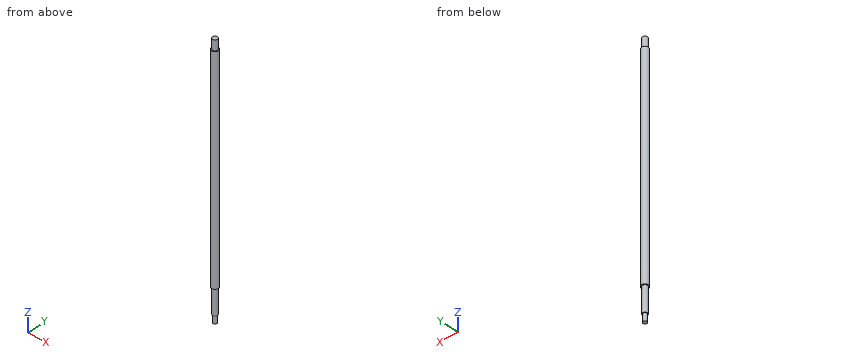
from build123d import *

# Parameters (mm, degrees)
SKETCH1_R           = 7
BOSS_EXTRUDE1_DEPTH = 431
SKETCH2_R           = 5
BOSS_EXTRUDE2_DEPTH = 20
BOSS_EXTRUDE3_START = 50
SKETCH3_R           = 5
BOSS_EXTRUDE3_DEPTH = 50
SKETCH4_R           = 4
BOSS_EXTRUDE4_DEPTH = 15


with BuildPart() as part:
    # Sketch1 → Boss-Extrude1 (new body)
    with BuildSketch(Plane.XY):
        Circle(SKETCH1_R)
    extrude(amount=BOSS_EXTRUDE1_DEPTH)

    # Sketch2 → Boss-Extrude2 (add)
    with BuildSketch(Plane.XY.offset(431)):
        Circle(SKETCH2_R)
    extrude(amount=BOSS_EXTRUDE2_DEPTH)

    # Sketch3 → Boss-Extrude3 (add)
    with BuildSketch(Plane(origin=(0, 0, 0), x_dir=(-1, 0, 0), z_dir=(0, 0, -1)).offset(BOSS_EXTRUDE3_START)):
        with Locations(Location((0, 0, 0), (0, 0, 180))):
            Circle(SKETCH3_R)
    extrude(amount=-BOSS_EXTRUDE3_DEPTH)

    # Sketch4 → Boss-Extrude4 (add)
    with BuildSketch(Plane(origin=(0, 0, -50), x_dir=(-1, 0, 0), z_dir=(0, 0, -1))):
        Circle(SKETCH4_R)
    extrude(amount=BOSS_EXTRUDE4_DEPTH)


solid = part.part
The listing builds one solid part. Answer for the finished solid, in the listing's coordinates (mm). Give positions to 0.01 mm unless a question says otherwise; leave off trailing zeros. Loops run counter-clockwise (first coordinate to the right, second up) from the corner with the lowest first, then second, coordinate; pieces in that order, holes last. Notation, with made-up numbers: (-24, -31) - (15, -31) arc R24 ccw to (15, -14) - close; hole circle Ø10 at (-23, 20). An arc over 180 degrees is marked (long way). Use one line per item in the form item = value.
1. Section A-A on x = 0 is taken. Give the vertices of the cut face in (y, z), then the cut area to 3 significant figures.
Calculated:
outline = (-7, 0) - (-5, 0) - (-5, -50) - (-4, -50) - (-4, -65) - (4, -65) - (4, -50) - (5, -50) - (5, 0) - (7, 0) - (7, 431) - (5, 431) - (5, 451) - (-5, 451) - (-5, 431) - (-7, 431) - close
area = 6,850 mm^2
2. Find the intervals of material crossed by line 1 along X through (y, z) = (1, 189); line 2 along Z through (x, y) = (-3.25, 5.25); line 3 along X through (y, z) = (-0.75, 287), in increasing order. Write a range as [from, to].
Calculated:
line_1 = [-6.93, 6.93]
line_2 = [0, 431]
line_3 = [-6.96, 6.96]
3. Section C-C on z = 341 is taken. Give the vertices of the cut face in (x, y), then the cut area to 3 significant figures.
Calculated:
outline = circle Ø14 at (0, 0)
area = 154 mm^2
4. Given pin 1 Ø4 at (x, z) = (-3.5, 282) entering from +Y; pin 2 Ø2 at (y, z) = (4.5, 109) entering from +X; pin 3 Ø3 at (y, z) = (-1, 181) entering from -X; pin 4 Ø2 at (y, z) = (3, 306) entering from +X, each flat-ended and moving along its own axis, determine where each tip first touches the part or whether it passes through.
Calculated:
pin_1 = 6.84
pin_2 = 6.06
pin_3 = -7
pin_4 = 6.71
